from build123d import *

# Parameters (mm, degrees)
SKETCH1_W           = 70
SKETCH1_H           = 30
BOSS_EXTRUDE1_DEPTH = 10
SKETCH8_R           = 5
CUT_EXTRUDE6_DEPTH  = 11
SKETCH9_R           = 6
CUT_EXTRUDE7_DEPTH  = 11
M4_TAPPED_HOLE2_D   = 3.3
SKETCH13_W          = 40
SKETCH13_H          = 10
BOSS_EXTRUDE2_DEPTH = 20
SKETCH14_R          = 2
CUT_EXTRUDE8_DEPTH  = 77.811457479
M3_TAPPED_HOLE1_D   = 2.5
CHAMFER3_SIZE       = 3
FILLET1_R           = 5
CHAMFER4_SIZE       = 0.5
SKETCH18_R          = 3.5
CUT_EXTRUDE9_DEPTH  = 2.5
CUT_EXTRUDE10_START = -2.5
SKETCH19_R          = 3.5
CUT_EXTRUDE10_DEPTH = 2.5


with BuildPart() as part:
    # Sketch1 → Boss-Extrude1 (new body)
    with BuildSketch(Plane(origin=(0, 0, 0), x_dir=(1, 0, 0), z_dir=(0, 1, 0))):
        with Locations((-35, 15)):
            Rectangle(SKETCH1_W, SKETCH1_H)
    extrude(amount=BOSS_EXTRUDE1_DEPTH)

    # Sketch8 → Cut-Extrude6 (cut)
    with BuildSketch(Plane.XZ):
        with Locations(Location((-13, -23, 0), (0, 0, 270))):
            Circle(SKETCH8_R)
    extrude(amount=-CUT_EXTRUDE6_DEPTH, mode=Mode.SUBTRACT)

    # Sketch9 → Cut-Extrude7 (cut)
    with BuildSketch(Plane.XZ):
        with Locations(Location((-60, -23, 0), (0, 0, 270))):
            Circle(SKETCH9_R)
        with Locations(Location((-35, -23, 0), (0, 0, 270))):
            Circle(SKETCH9_R)
    extrude(amount=-CUT_EXTRUDE7_DEPTH, mode=Mode.SUBTRACT)

    # M4 Tapped Hole2 (through all)
    with Locations(Plane(origin=(0, 0, 0), x_dir=(-1, 0, 0), z_dir=(0, -1, 0))):
        with Locations((65, 5), (5, 5)):
            Hole(M4_TAPPED_HOLE2_D / 2)

    # Sketch13 → Boss-Extrude2 (add)
    with BuildSketch(Plane.XY):
        with Locations((-35, 5)):
            Rectangle(SKETCH13_W, SKETCH13_H)
    extrude(amount=BOSS_EXTRUDE2_DEPTH)

    # Sketch14 → Cut-Extrude8 (cut, through all)
    with BuildSketch(Plane(origin=(0, 10, 0), x_dir=(1, 0, 0), z_dir=(0, 1, 0))):
        with Locations(Location((-50, -10.5, 0), (0, 0, 270))):
            Circle(SKETCH14_R)
        with Locations(Location((-20, -10.5, 0), (0, 0, 270))):
            Circle(SKETCH14_R)
    extrude(amount=-CUT_EXTRUDE8_DEPTH, mode=Mode.SUBTRACT)

    # M3 Tapped Hole1 (through all)
    with Locations(Plane(origin=(0, 0, 0), x_dir=(-1, 0, 0), z_dir=(0, -1, 0))):
        with Locations((25, 2.5), (45, 2.5)):
            Hole(M3_TAPPED_HOLE1_D / 2)

    # Chamfer3
    chamfer3_edges = [part.edges().sort_by_distance(p)[0] for p in [
        (0, 5, -30),
        (0, 5, 0),
        (-15, 5, 20),
        (-55, 5, 20),
        (-70, 5, 0),
        (-70, 5, -30),
    ]]
    chamfer(chamfer3_edges, length=CHAMFER3_SIZE)

    # Fillet1
    fillet1_edges = [part.edges().sort_by_distance(p)[0] for p in [
        (-15, 5, 0),
        (-55, 5, 0),
    ]]
    fillet(fillet1_edges, radius=FILLET1_R)

    # Chamfer4
    chamfer4_edges = [part.edges().sort_by_distance(p)[0] for p in [
        (-6.5, 0, 0),
        (-6.5, 10, 0),
        (-13.535533906, 10, 1.464466094),
        (-13.535533906, 0, 1.464466094),
        (-56.464466094, 0, 1.464466094),
        (-56.464466094, 10, 1.464466094),
        (-35, 0, -30),
        (-35, 10, -30),
        (-70, 0, -15),
        (0, 0, -15),
        (-15, 0, 11),
        (-35, 0, 20),
        (-55, 0, 11),
        (-63.5, 0, 0),
        (0, 10, -15),
        (-70, 10, -15),
        (-63.5, 10, 0),
        (-55, 10, 11),
        (-35, 10, 20),
        (-15, 10, 11),
    ]]
    chamfer(chamfer4_edges, length=CHAMFER4_SIZE)

    # Sketch18 → Cut-Extrude9 (cut)
    with BuildSketch(Plane(origin=(0, 10, 0), x_dir=(1, 0, 0), z_dir=(0, 1, 0))):
        with Locations(Location((-50, -10.5, 0), (0, 0, 270))):
            Circle(SKETCH18_R)
        with Locations(Location((-20, -10.5, 0), (0, 0, 270))):
            Circle(SKETCH18_R)
    extrude(amount=-CUT_EXTRUDE9_DEPTH, mode=Mode.SUBTRACT)

    # Sketch19 → Cut-Extrude10 (cut)
    with BuildSketch(Plane.XZ.offset(CUT_EXTRUDE10_START)):
        with Locations(Location((-50, 10.5, 0), (0, 0, 90))):
            Circle(SKETCH19_R)
        with Locations(Location((-20, 10.5, 0), (0, 0, 90))):
            Circle(SKETCH19_R)
    extrude(amount=CUT_EXTRUDE10_DEPTH, mode=Mode.SUBTRACT)


solid = part.part
Source: CAD feature listing. Evaluate the final solid. Frame: model axes, mm. A direction names the side the tool comes from. Coordinates: 2 decimals unless noted, no trailing zeros. Order: outer loops, then holes, each group sorted by start corner. A loop starts at its lowest first (then second) coordinate and runs counter-clockwise, first axis right, second up.
Item 1: Material intervals for line 1 (X direction, y = 4, z = -5); line 2 (X direction, y = 9.35, z = 10.5); line 3 (Z direction, x = -65, y = 4.5), sorted ascending.
Output values:
line 1: x = -70 to -66.65, -63.35 to -6.65, -3.35 to 0
line 2: x = -55 to -53.5, -46.5 to -23.5, -16.5 to -15
line 3: z = -30 to -26.32, -19.68 to -6.65, -3.35 to 0
Item 2: Set-up query: faces 1 (the face through (-22.365, 1.268, 7.92)), 2 (the face through (-52, 7.5, 12)), 3 (the face through (-15, 5, 11)), 4 (the face through (-46.25, 5.07, -2.55)). Return all of +Z, -Z, +X, -X, +Y, -Y with unobstructed straight access to the full face (end or side cutting, diameter ignored); none if empty.
Output values:
face 1: -Y
face 2: +Y
face 3: +Z, +X, +Y, -Y
face 4: +Y, -Y
Item 3: Cut plane C-C (z = -5). Return loops of the section in (x, y), plus the area to 4 significant figures.
Output values:
outline: (-70, 0.5) - (-69.5, 0) - (-66.65, 0) - (-66.65, 10) - (-69.5, 10) - (-70, 9.5) - close; (-63.35, 0) - (-6.65, 0) - (-6.65, 10) - (-63.35, 10) - close; (-3.35, 0) - (-0.5, 0) - (0, 0.5) - (0, 9.5) - (-0.5, 10) - (-3.35, 10) - close
area: 633.5 mm2
Item 4: First-contact query: P1, Ø3, axis at x = -5, z = -5, coming from the -Y side; P2, Ø2.5, axis at y = 5, z = 8.5, coming from the -X side; P3, Ø5, axis at x = -58.5, y = 3, coming from the +Z side; P4, Ø4.5, axis at x = -20, z = 10.5, coming from the +Y side. Flat tips, straight axial feed; report the tip coordinate or a pass-through.
Output values:
P1: passes through
P2: stops at x = -55
P3: stops at z = 2
P4: stops at y = 7.5
Item 5: Pull-direction query (X, two-part tool) for faces 5 (the face through (-53.47, 1.27, 10.04)), 6 (the face through (-13.671, 0.365, 1.409)), 7 (the face through (-48, 2.5, 12)), 8 (the face through (-57, 5, 1)); classes: pulls with the +X half, pulls with the -X half, needs draft (parallel to the pull), parting line crosses it, or undercut.
Output values:
face 5: undercut
face 6: pulls with the +X half
face 7: undercut
face 8: pulls with the -X half
Item 6: Cut plane A-A (y = 5.25). Count the separate pieces of the cut face and the enclosed holes in it, plus the area to 3 significant figures.
Output values:
separate pieces: 1
enclosed holes: 9
area: 2,530 mm2
Item 7: Cut plane B-B (x = -20). Return loops of the section in (y, z), plus the area to 4 significant figures.
Output values:
outline: (0, -29.5) - (0.5, -30) - (9.5, -30) - (10, -29.5) - (10, 7) - (7.5, 7) - (7.5, 8.5) - (2.5, 8.5) - (2.5, 7) - (0, 7) - close; (0, 14) - (2.5, 14) - (2.5, 12.5) - (7.5, 12.5) - (7.5, 14) - (10, 14) - (10, 19.5) - (9.5, 20) - (0.5, 20) - (0, 19.5) - close
area: 444.5 mm2
Item 8: Cut plane D-D (z = -22.5). Return loops of the section in (x, y), plus the area to 3 significant figures.
Output values:
outline: (-70, 0.5) - (-69.5, 0) - (-65.98, 0) - (-65.98, 10) - (-69.5, 10) - (-70, 9.5) - close; (-54.02, 0) - (-40.98, 0) - (-40.98, 10) - (-54.02, 10) - close; (-29.02, 0) - (-17.97, 0) - (-17.97, 10) - (-29.02, 10) - close; (-8.03, 0) - (-0.5, 0) - (0, 0.5) - (0, 9.5) - (-0.5, 10) - (-8.03, 10) - close
area: 361 mm2
